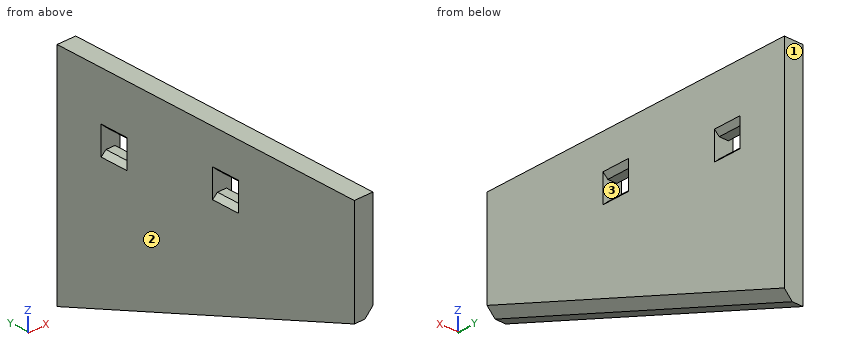
from build123d import *

# Parameters (mm, degrees)
BOSS_EXTRUDE1_DEPTH = 17.5
CUT_EXTRUDE1_START  = 185
CUT_EXTRUDE1_DEPTH  = 26
CHAMFER2_SIZE       = 15
CUT_EXTRUDE2_START  = -40
CUT_EXTRUDE2_DEPTH  = 26


with BuildPart() as part:
    # Sketch1 → Boss-Extrude1 (new, symmetric)
    with BuildSketch(Plane(origin=(0, 0, 0), x_dir=(0, 0, -1), z_dir=(1, 0, 0))):
        Polygon((0, 0), (0, 300), (413, 300), (194.61785944, -300), (0, -300), align=None)
    extrude(amount=BOSS_EXTRUDE1_DEPTH, both=True)

    # Sketch2 → Cut-Extrude1 (cut, symmetric)
    with BuildSketch(Plane(origin=(0, 0, 0), x_dir=(1, 0, 0), z_dir=(0, 1, 0)).offset(CUT_EXTRUDE1_START)):
        Polygon((-17.5, 89), (-8.5, 97.5), (8.5, 97.5), (17.5, 89), (17.5, 141), (8.5, 132.5), (-8.5, 132.5), (-17.5, 141), align=None)
    extrude(amount=CUT_EXTRUDE1_DEPTH, both=True, mode=Mode.SUBTRACT)

    # Chamfer2
    chamfer2_edges = [part.edges().sort_by_distance(p)[0] for p in [
        (17.5, 0, -303.80892972),
    ]]
    chamfer(chamfer2_edges, length=CHAMFER2_SIZE)

    # Sketch3 → Cut-Extrude2 (cut, symmetric)
    with BuildSketch(Plane(origin=(0, 0, 0), x_dir=(1, 0, 0), z_dir=(0, 1, 0)).offset(CUT_EXTRUDE2_START)):
        Polygon((-17.5, 64), (-8.5, 72.5), (8.5, 72.5), (17.5, 64), (17.5, 116), (8.5, 107.5), (-8.5, 107.5), (-17.5, 116), align=None)
    extrude(amount=CUT_EXTRUDE2_DEPTH, both=True, mode=Mode.SUBTRACT)


solid = part.part
Here's how the part is built. I have some questions about the finished solid (model axes, mm). Face numbers are marked on the shaded views. Give positions to 0.01 mm unless a question says otherwise; leave off trailing zeros. Loops run counter-clockwise (first coordinate to the right, second up) from the corner with the lowest first, then second, coordinate; pieces in that order, holes last. Notation, with made-up numbers: (60, 87.5) -> (65, 87.5) arc R23 cw to (65, 125.5) -> close; hole circle Ø1 at (-37.75, 59). An arc over 180 degrees is marked (long way). Answer as a JSON object with one key per item and string values. Group by question number.
Item 1: Will these pins go through, and if not, where does the flat tip stop? pin 1 (13.5 mm diameter, centred on x = -1, y = -41, fed in from -Z); pin 2 (5 mm diameter, centred on x = -3.5, y = 188, fed in from +Z); pin 3 (2 mm diameter, centred on x = 11, y = 182.5, fed in from -Z); pin 4 (12 mm diameter, centred on x = -7, y = 92, fed in from -Z).
Item 2: I need wall thicknesses on L1, parallel to Y at x = -0.5, z = -90; L2, parallel to Z at x = 2, y = -40.5; L3, parallel to Z at x = -4.5, y = -155. Which ranges of each line are inside material? Lowest first, please.
Item 3: Imagine slicing it at B-B on y = 139. Write out the boundary of the cut face in (x, z), then the cut area to 3 significant figures.
Item 4: Thinking about a two-plate mould opening in Y: for the marked faces 1, 2 and 3, which applies, pulls with the +Y half, pulls with the -Y half, needs draft (parallel to the pull), parting line crosses it, or undercut?
Item 5: Imagine slicing it at C-C on z = -368. Write out the boundary of the cut face in (x, y).
Item 6: Imagine slicing it at A-A on z = -126.5. Write out the boundary of the cut face in (x, y), then the cut area to 3 significant figures.
Answer list:
{
 "1": {"pin 1": "stops at z = -291.34", "pin 2": "stops at z = 0", "pin 3": "stops at z = -362.31", "pin 4": "stops at z = -339.48"},
 "2": {"L1": "y = -300 to -66, -14 to 300", "L2": "z = -289.07 to -107.5, -72.5 to 0", "L3": "z = -247.39 to 0"},
 "3": {"outline": "(-17.5, -354.4) -> (2.5, -354.4) -> (17.5, -338.44) -> (17.5, 0) -> (-17.5, 0) -> close", "area": "12,300 mm2"},
 "4": {"face 1": "pulls with the +Y half", "face 2": "needs draft", "face 3": "undercut"},
 "5": {"outline": "(-17.5, 176.36) -> (2.5, 176.36) -> (17.5, 220.22) -> (17.5, 300) -> (-17.5, 300) -> close"},
 "6": {"outline": "(-17.5, -300) -> (17.5, -300) -> (17.5, 159) -> (-17.5, 159) -> close; (-17.5, 211) -> (17.5, 211) -> (17.5, 300) -> (-17.5, 300) -> close", "area": "19,200 mm2"}
}
